Source: CAD feature listing. Evaluate the final solid. Frame: model axes, mm. A direction names the side the tool comes from. Give positions to 0.01 mm unless a question says otherwise; leave off trailing zeros. Loops run counter-clockwise (first coordinate to the right, second up) from the corner with the lowest first, then second, coordinate; pieces in that order, holes last. Notation, with made-up numbers: M 80.25,58.5 L 126.25,58.5 A26 cw 126.25,82.5 Z; hole C 50,-13 d6. An arc over 180 degrees is marked long. Answer in a Markdown table with one row per item.
```python
from build123d import *

# Parameters (mm, degrees)
HUB_PROFILE_SKETCH_R   = 30
HUB_PROFILE_SKETCH_R_2 = 15
HUB_60_BORE_30_DEPTH   = 25
LEVER_ARM_WEB_DEPTH    = 5
CLEVIS_LUG_SKETCH_R    = 6
CLEVIS_LUG_DEPTH       = 9


with BuildPart() as part:
    # Hub Profile Sketch → Hub Ø60 Bore Ø30 (new, symmetric)
    with BuildSketch(Plane.XY):
        Circle(HUB_PROFILE_SKETCH_R)
        Circle(HUB_PROFILE_SKETCH_R_2, mode=Mode.SUBTRACT)
    extrude(amount=HUB_60_BORE_30_DEPTH, both=True)

    # Lever Arm Sketch → Lever Arm Web (add, symmetric)
    with BuildSketch(Plane.XY):
        with BuildLine():
            Line((4.671688756, 29.634023084), (97.5, 15))
            Line((97.5, 15), (122.5, 15))
            Line((122.5, 15), (122.5, -15))
            Line((122.5, -15), (97.5, -15))
            Line((97.5, -15), (4.671688756, -29.634023084))
            ThreePointArc((4.671688756, -29.634023084), (30, 0), (4.671688756, 29.634023084))
        make_face()
    extrude(amount=LEVER_ARM_WEB_DEPTH, both=True)

    # Clevis Lug Sketch → Clevis Lug (add)
    with BuildSketch(Plane.XZ.offset(15)):
        with BuildLine():
            Line((97.5, 5), (97.5, 20))
            ThreePointArc((97.5, 20), (110, 32.5), (122.5, 20))
            Line((122.5, 20), (122.5, 5))
            Line((122.5, 5), (97.5, 5))
        make_face()
        with Locations((110, 20)):
            Circle(CLEVIS_LUG_SKETCH_R, mode=Mode.SUBTRACT)
    clevis_lug = extrude(amount=-CLEVIS_LUG_DEPTH)

    # Clevis Lug Mirror: Clevis Lug across plane
    add(clevis_lug.mirror(Plane.ZX))


solid = part.part
```
1) Section D-D, the plane x = 9.5. Return loops of the section in (y, z), then the cut area to 3 significant figures.
Reply:
| item | result |
|---|---|
| outline | M -28.87,-5 L -28.46,-5 L -28.46,-25 L -11.61,-25 L -11.61,25 L -28.46,25 L -28.46,5 L -28.87,5 Z; M 11.61,-25 L 28.46,-25 L 28.46,-5 L 28.87,-5 L 28.87,5 L 28.46,5 L 28.46,25 L 11.61,25 Z |
| area | 1,690 mm² |
2) Material intervals for L1, parallel to Y at x = 0, z = 6; L2, parallel to Z at x = 110, y = 13; L3, parallel to Z at x = 26.5, y = 24, sorted ascending.
Reply:
| item | result |
|---|---|
| L1 | y = -30 to -15, 15 to 30 |
| L2 | z = -5 to 14, 26 to 32.5 |
| L3 | z = -5 to 5 |
3) Section A-A, the plane x = 110. Return loops of the section in (y, z).
Reply:
| item | result |
|---|---|
| outline | M -15,-5 L 15,-5 L 15,14 L 6,14 L 6,5 L -6,5 L -6,14 L -15,14 Z; M -15,26 L -6,26 L -6,32.5 L -15,32.5 Z; M 6,26 L 15,26 L 15,32.5 L 6,32.5 Z |
4) Set-up query: faces 5 (the flat face through (110, 15, 10)), 6 (the cylindrical face through (-29.97, 1.32, 0.35)), 7 (the flat face through (97.5, -11, 12)), 8 (the flat face through (110, -15, 10)), 9 (the flat face through (110, -6, 13)). Return all of +Z, -Z, +X, -X, +Y, -Y with unobstructed straight access to the full face (end or side cutting, diameter ignored); none if empty.
Reply:
| item | result |
|---|---|
| face 5 | +Z, -Z, +X, +Y |
| face 6 | none |
| face 7 | +Z, +Y, -Y |
| face 8 | +Z, -Z, +X, -Y |
| face 9 | +Z, +X |
5) Pull-direction query (X, two-part tool) for faces 1 (the flat face through (6, 14, -25)), 2 (the cylindrical face through (-14.985, 0.66, -0.35)), 3 (the flat face through (122.5, 0, 2)), 4 (the flat face through (97.5, 11, 12)); classes: released by +X, released by -X, zero draft, split by the parting line, or undercut.
Reply:
| item | result |
|---|---|
| face 1 | zero draft |
| face 2 | undercut |
| face 3 | released by +X |
| face 4 | undercut |
6) Pin query (flat end, axial travel): pin 1 Ø1.5 at (y, z) = (5, 6) entering from +X; pin 2 Ø7.5 at (x, z) = (108, 10.5) entering from -Y; pin 3 Ø7.5 at (x, z) = (107.5, 25) entering from +Y. Return the tip coordinate at first contact, or that it passes through.
Reply:
| item | result |
|---|---|
| pin 1 | stops at x = 29.7 |
| pin 2 | stops at y = -15 |
| pin 3 | stops at y = 15 |
7) Section B-B, the plane z = 12. Return loops of the section in (x, y).
Reply:
| item | result |
|---|---|
| outline | C 0,0 d60; M 97.5,-15 L 122.5,-15 L 122.5,-6 L 97.5,-6 Z; M 97.5,6 L 122.5,6 L 122.5,15 L 97.5,15 Z; hole C 0,0 d30 |
8) Section C-C, the plane y = 0. Return loops of the section in (x, z).
Reply:
| item | result |
|---|---|
| outline | M -30,-25 L -15,-25 L -15,25 L -30,25 Z; M 15,-25 L 30,-25 L 30,-5 L 122.5,-5 L 122.5,5 L 30,5 L 30,25 L 15,25 Z |
